```python
from build123d import *

# Parameters (mm, degrees)
BOSS_EXTRUDE1_DEPTH                                  = 10
SKETCH2_R                                            = 14
CUT_EXTRUDE1_DEPTH                                   = 128.671453348
M4_TAPPED_HOLE1_D                                    = 3.3
CBORE_FOR_M6_HEXAGON_SOCKET_HEAD_CAP_SCR_D           = 6.6
CBORE_FOR_M6_HEXAGON_SOCKET_HEAD_CAP_SCR_CBORE_D     = 11
CBORE_FOR_M6_HEXAGON_SOCKET_HEAD_CAP_SCR_CBORE_DEPTH = 6.8
CHAMFER1_SIZE                                        = 2
FILLET1_R                                            = 3


with BuildPart() as part:
    # Sketch1 → Boss-Extrude1 (new body)
    with BuildSketch(Plane.XY):
        Polygon((-90, 55), (-50, 55), (-50, -55), (-90, -55), (-90, -90), (-55, -90), (-55, -70), (55, -70), (55, -90), (90, -90), (90, -55), (50, -55), (50, 55), (90, 55), (90, 90), (55, 90), (55, 70), (-55, 70), (-55, 90), (-90, 90), align=None)
    extrude(amount=BOSS_EXTRUDE1_DEPTH)

    # Sketch2 → Cut-Extrude1 (cut, through all)
    with BuildSketch(Plane(origin=(0, 0, 0), x_dir=(-1, 0, 0), z_dir=(0, 0, -1))):
        Circle(SKETCH2_R)
    extrude(amount=-CUT_EXTRUDE1_DEPTH, mode=Mode.SUBTRACT)

    # M4 Tapped Hole1 (through all)
    with Locations(Plane.XY.offset(10)):
        with Locations((25, -55)):
            Hole(M4_TAPPED_HOLE1_D / 2)

    # CBORE for M6 Hexagon socket head cap screws1 (through all)
    with Locations(Plane(origin=(0, 0, 0), x_dir=(-1, 0, 0), z_dir=(0, 0, -1))):
        with Locations((78, -75), (78, 75), (-81.36030205, 75), (-81.36030205, -75)):
            CounterBoreHole(CBORE_FOR_M6_HEXAGON_SOCKET_HEAD_CAP_SCR_D / 2, CBORE_FOR_M6_HEXAGON_SOCKET_HEAD_CAP_SCR_CBORE_D / 2, CBORE_FOR_M6_HEXAGON_SOCKET_HEAD_CAP_SCR_CBORE_DEPTH)

    # Chamfer1
    chamfer1_edges = [part.edges().sort_by_distance(p)[0] for p in [
        (-90, 55, 5),
        (-90, 90, 5),
        (-55, 90, 5),
        (55, 90, 5),
        (90, 90, 5),
        (90, 55, 5),
        (90, -55, 5),
        (90, -90, 5),
        (55, -90, 5),
        (-55, -90, 5),
        (-90, -90, 5),
        (-90, -55, 5),
    ]]
    chamfer(chamfer1_edges, length=CHAMFER1_SIZE)

    # Fillet1
    fillet1_edges = [part.edges().sort_by_distance(p)[0] for p in [
        (-55, 70, 5),
        (55, 70, 5),
        (50, 55, 5),
        (50, -55, 5),
        (55, -70, 5),
        (-55, -70, 5),
        (-50, -55, 5),
        (-50, 55, 5),
    ]]
    fillet(fillet1_edges, radius=FILLET1_R)


solid = part.part
```
The model under review builds one solid part; all positions refer to its coordinate system, in mm. A direction names the side the tool comes from. Coordinates: 2 decimals unless noted, no trailing zeros. Write each loop counter-clockwise with the first axis right and the second up, starting at its lowest first coordinate (ties: lowest second). Pieces come first, ordered by that corner, then holes. Notation, with made-up numbers: (-3, 72) - (28, 72) arc R30 ccw to (28, 110) - close; hole circle Ø10 at (77, -25.5). An arc over 180 degrees is marked (long way). Answer in a Markdown table with one row per item. Add a question column.
Q1. For faces 4 (the face through (70, 55, 5)), 5 (the face through (-73.95, -71.28, 3.35)), 6 (the face through (-70, -55, 5)), 7 (the face through (55, -80, 5)), 8 (the face through (-55, 80, 5)), list the 3-axis set-ups (+Z, -Z, +X, -X, +Y, -Y) from which the entire face can be reached by the end or side of a thin tool; tool diameter is ignored.
Q2. Draft analysis for pull direction Y (two halves, no side actions). For faces 1 (the face through (-1, 21, 0)), 2 (the face through (73, 90, 5)), 3 (the face through (83.134, 77.783, 8.422)), state which applies: +Y half, -Y half, draft (parallel to the pull), parting line (faces both ways), or undercut.
Q3. Consider section D-D on y = 46. Give the boundary of the cut face in (x, z).
Q4. Consider section B-B on y = -11. Give the boundary of the cut face in (x, z).
Q5. Consider section A-A on x = 0. Give the boundary of the cut face in (y, z).
Q6. To check wall thickness, follow line 1 along Y through (x, z) = (-78, 3.75); line 2 along Y through (x, z) = (-78, 7.6); line 3 along Y through (x, z) = (25, 5.5). State the ranges of each line that lie inside material, in increasing order. Write a range as from..to.
Q7. Consider section C-C on z = 3. Give the number of separate pieces and of enclosed holes in the cut face, then the cut area to 3 significant figures.
Q8. Clearance check with flat-ended pins moving along their axes: pin 1 (9 mm diameter, centred on x = -78, y = -75, fed in from -Z); pin 2 (3 mm diameter, centred on y = 38, z = 2, fed in from +X); pin 3 (4 mm diameter, centred on x = 11, z = 8, fed in from +Y). State where each tip first meets the part, or that it passes through.
Answers below:
| question | item | result |
|---|---|---|
| 1 | face 4 | +Z, -Z, +X |
| 1 | face 5 | -Z |
| 1 | face 6 | +Z, -Z, -X |
| 1 | face 7 | +Z, -Z, -Y |
| 1 | face 8 | +Z, -Z, +Y |
| 2 | face 1 | draft |
| 2 | face 2 | +Y half |
| 2 | face 3 | undercut |
| 3 | outline | (-50, 0) - (50, 0) - (50, 10) - (-50, 10) - close |
| 4 | outline | (-50, 0) - (-8.66, 0) - (-8.66, 10) - (-50, 10) - close; (8.66, 0) - (50, 0) - (50, 10) - (8.66, 10) - close |
| 5 | outline | (-70, 0) - (-14, 0) - (-14, 10) - (-70, 10) - close; (14, 0) - (70, 0) - (70, 10) - (14, 10) - close |
| 6 | line 1 | -90..-80.5, -69.5..-55, 55..69.5, 80.5..90 |
| 6 | line 2 | -90..-78.3, -71.7..-55, 55..71.7, 78.3..90 |
| 6 | line 3 | -70..-56.65, -53.35..70 |
| 7 | separate pieces | 1 |
| 7 | enclosed holes | 6 |
| 7 | area | 18,200 mm² |
| 8 | pin 1 | z = 6.8 |
| 8 | pin 2 | x = 50 |
| 8 | pin 3 | y = 70 |
